```python
from build123d import *

# Parameters (mm, degrees)
SKETCH1_W                    = 16
SKETCH1_H                    = 55
BOSS_EXTRUDE1_DEPTH          = 3
CUT_EXTRUDE2_DEPTH           = 10
SKETCH5_W                    = 6
SKETCH5_H                    = 20
CUT_EXTRUDE3_DEPTH           = 10
FILLET1_R                    = 2.5
CHAMFER1_SIZE                = 1
CHAMFER2_SIZE                = 0.5
M2_TAPPED_HOLE1_D            = 1.6
M2_TAPPED_HOLE1_DEPTH        = 5.2
M2_TAPPED_HOLE1_TIP          = 0.480688495
F_4_0_4_DIAMETER_HOLE1_D     = 4
F_4_0_4_DIAMETER_HOLE1_DEPTH = 4
F_4_0_4_DIAMETER_HOLE1_TIP   = 1.201721238


with BuildPart() as part:
    # Sketch1 → Boss-Extrude1 (new body)
    with BuildSketch(Plane(origin=(0, 0, 0), x_dir=(1, 0, 0), z_dir=(0, 1, 0))):
        with Locations((8, -27.5)):
            Rectangle(SKETCH1_W, SKETCH1_H)
    extrude(amount=BOSS_EXTRUDE1_DEPTH)

    # Sketch4 → Cut-Extrude2 (cut)
    with BuildSketch(Plane.XZ):
        with BuildLine():
            Line((5.1, 51.5), (5.1, 46.5))
            ThreePointArc((5.1, 46.5), (3.5, 44.9), (1.9, 46.5))
            Line((1.9, 46.5), (1.9, 51.5))
            ThreePointArc((1.9, 51.5), (3.5, 53.1), (5.1, 51.5))
        make_face()
        with BuildLine():
            Line((10.9, 51.5), (10.9, 46.5))
            ThreePointArc((10.9, 46.5), (12.5, 44.9), (14.1, 46.5))
            Line((14.1, 46.5), (14.1, 51.5))
            ThreePointArc((14.1, 51.5), (12.5, 53.1), (10.9, 51.5))
        make_face()
    extrude(amount=-CUT_EXTRUDE2_DEPTH, mode=Mode.SUBTRACT)

    # Sketch5 → Cut-Extrude3 (cut)
    with BuildSketch(Plane(origin=(0, 3, 0), x_dir=(1, 0, 0), z_dir=(0, 1, 0))):
        with Locations((3, -10)):
            Rectangle(SKETCH5_W, SKETCH5_H)
    extrude(amount=-CUT_EXTRUDE3_DEPTH, mode=Mode.SUBTRACT)

    # Fillet1
    fillet1_edges = [part.edges().sort_by_distance(p)[0] for p in [
        (6, 1.5, 20),
    ]]
    fillet(fillet1_edges, radius=FILLET1_R)

    # Chamfer1
    chamfer1_edges = [part.edges().sort_by_distance(p)[0] for p in [
        (0, 1.5, 20),
        (6, 1.5, 0),
        (16, 1.5, 0),
        (16, 1.5, 55),
        (0, 1.5, 55),
    ]]
    chamfer(chamfer1_edges, length=CHAMFER1_SIZE)

    # Chamfer2
    chamfer2_edges = [part.edges().sort_by_distance(p)[0] for p in [
        (0, 3, 37.5),
        (16, 3, 27.5),
    ]]
    chamfer(chamfer2_edges, length=CHAMFER2_SIZE)

    # M2 Tapped Hole1
    with Locations(Plane(origin=(0, 3, 0), x_dir=(1, 0, 0), z_dir=(0, 1, 0))):
        with Locations((13.5, -3.25), (13.5, -14.25)):
            Hole(M2_TAPPED_HOLE1_D / 2, depth=M2_TAPPED_HOLE1_DEPTH)
            with Locations((0, 0, -(M2_TAPPED_HOLE1_DEPTH + M2_TAPPED_HOLE1_TIP / 2))):  # 118° drill point
                Cone(0, M2_TAPPED_HOLE1_D / 2, M2_TAPPED_HOLE1_TIP, mode=Mode.SUBTRACT)

    # Ø4.0 (4) Diameter Hole1
    with Locations(Plane(origin=(0, 0, 0), x_dir=(-1, 0, 0), z_dir=(0, -1, 0))):
        with Locations((-8, -35)):
            Hole(F_4_0_4_DIAMETER_HOLE1_D / 2, depth=F_4_0_4_DIAMETER_HOLE1_DEPTH)
            with Locations((0, 0, -(F_4_0_4_DIAMETER_HOLE1_DEPTH + F_4_0_4_DIAMETER_HOLE1_TIP / 2))):  # 118° drill point
                Cone(0, F_4_0_4_DIAMETER_HOLE1_D / 2, F_4_0_4_DIAMETER_HOLE1_TIP, mode=Mode.SUBTRACT)


solid = part.part
```
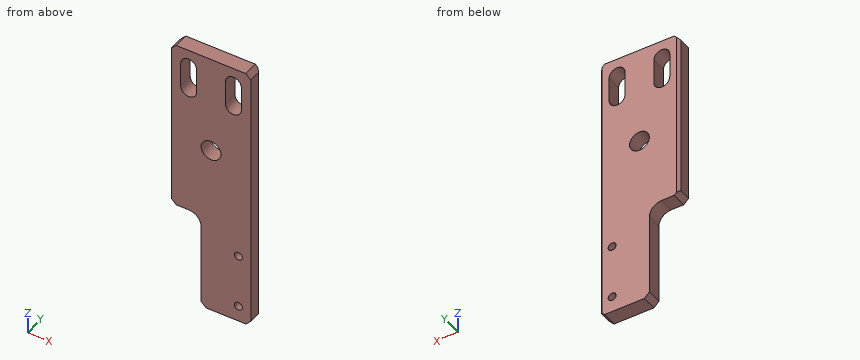
The model under review builds one solid part; all positions refer to its coordinate system, in mm. Round coordinates to 2 decimals unless told otherwise and drop trailing zeros. Write each loop counter-clockwise with the first axis right and the second up, starting at its lowest first coordinate (ties: lowest second). Pieces come first, ordered by that corner, then holes. Notation, with made-up numbers: (40, -4) - (96, -4) arc R6 cw to (96, 6) - close; hole circle Ø7 at (-20.75, 21.25). An arc over 180 degrees is marked (long way). Answer as CSV lines item,"result". Start each with the question number.
(1) We need section D-D on x = 13.5. State the section outline as (y, z) points, plus the area to 3 significant figures.
(2) We need section A-A on z = 14.25. State the section outline as (x, y) points.
(3) We need section C-C on x = 8. State the section outline as (y, z) points.
(4) We need section B-B on y = 0.8. State the section outline as (x, z) points.
(5) To check wall thickness, follow line 1 (X direction, y = 2.05, z = 14.25); line 2 (Z direction, x = 13.5, y = 1.05); line 3 (X direction, y = 1.2, z = 35). State the ranges of each line that lie inside material, in increasing order.
(6) For pin 1 Ø1.4 at (x, z) = (13.5, 3.25) entering from +Y; pin 2 Ø1.5 at (y, z) = (1, 6) entering from -X, all flat-tipped, find the tip position at first contact; note any pin that passes through.
Worked answers:
1,outline,"(0, 0) - (3, 0) - (3, 2.45) - (0, 2.45) - close; (0, 4.05) - (3, 4.05) - (3, 13.45) - (0, 13.45) - close; (0, 15.05) - (3, 15.05) - (3, 45.25) - (0, 45.25) - close; (0, 52.75) - (3, 52.75) - (3, 55) - (0, 55) - close"
1,area,"133 mm²"
2,outline,"(6, 0) - (12.7, 0) - (12.7, 3) - (6, 3) - close; (14.3, 0) - (16, 0) - (16, 2.5) - (15.5, 3) - (14.3, 3) - close"
3,outline,"(0, 0) - (3, 0) - (3, 33) - (0, 33) - close; (0, 37) - (3, 37) - (3, 55) - (0, 55) - close"
4,outline,"(0, 21) - (1, 20) - (3.5, 20) arc R2.5 cw to (6, 17.5) - (6, 1) - (7, 0) - (15, 0) - (16, 1) - (16, 54) - (15, 55) - (1, 55) - (0, 54) - close; hole (1.9, 46.5) arc R1.6 ccw to (5.1, 46.5) - (5.1, 51.5) arc R1.6 ccw to (1.9, 51.5) - close; hole circle Ø4 at (8, 35); hole (10.9, 46.5) arc R1.6 ccw to (14.1, 46.5) - (14.1, 51.5) arc R1.6 ccw to (10.9, 51.5) - close; hole circle Ø1.6 at (13.5, 3.25); hole circle Ø1.6 at (13.5, 14.25)"
5,line 1,"6 to 12.7, 14.3 to 16"
5,line 2,"0 to 2.45, 4.05 to 13.45, 15.05 to 45.25, 52.75 to 55"
5,line 3,"0 to 6, 10 to 16"
6,pin 1,"through"
6,pin 2,"x = 6"
